The model under review builds one solid part; all positions refer to its coordinate system, in mm. A direction names the side the tool comes from. Round coordinates to 2 decimals unless told otherwise and drop trailing zeros. Order: outer loops, then holes, each group sorted by start corner. A loop starts at its lowest first (then second) coordinate and runs counter-clockwise, first axis right, second up.
1) Machinability: for faces 1 (the face through (75, 22, -3.5)), 2 (the face through (170.645, 0.454, 0.049)), which of the approach directions +Z, -Z, +X, -X, +Y, -Y give a long, thin tool a straight path to every point of the face, cutting with its end or side? Answer none if there is none.
2) To check wall thickness, follow L1, parallel to Y at x = 29.5, z = 3; L2, parallel to X at y = 0.5, z = 0. State the ranges of each line that lie inside material, in increasing order.
3) Consider section B-B (x = 38.5). Give the boundary of the cut face in (y, z).
4) Consider section C-C (z = -0.5). Give the boundary of the cut face in (x, y).
5) Consider section A-A (y = 0). Give the boundary of the cut face in (x, z), then the cut area to 3 significant figures.
6) Clearance check with a flat-ended pin moving along its axis: P1, Ø2, axis at y = -3.5, z = 2, coming from the -X side. State where the tip first meets the part, or that it passes through.
7) Mouldability with a two-part tool opening along X and no side actions: class faces 3 (the face through (76, -20.65, 0)), 4 (the face through (-22.645, -0.498, 0.049)), 5 (the face through (-20.645, -0.454, 0.049)), 6 (the face through (74, 22.65, 0)) as pulls with the +X half, pulls with the -X half, needs draft (parallel to the pull), parting line crosses it, or undercut.
from build123d import *

# Parameters (mm, degrees)
EXTRUDE_1_DEPTH = 3.5


with BuildPart() as part:
    # 草图1 → 拉伸-薄壁1 (new, symmetric)
    with BuildSketch(Plane.XY):
        with BuildLine():
            Line((150, -22.65), (0, -22.65))
            ThreePointArc((0, -22.65), (-22.65, 0), (0, 22.65))
            Line((0, 22.65), (150, 22.65))
            ThreePointArc((150, 22.65), (172.65, 0), (150, -22.65))
        make_face()
        with BuildLine():
            Line((150, -20.65), (0, -20.65))
            ThreePointArc((0, -20.65), (-20.65, 0), (0, 20.65))
            Line((0, 20.65), (150, 20.65))
            ThreePointArc((150, 20.65), (170.65, 0), (150, -20.65))
        make_face(mode=Mode.SUBTRACT)
    extrude(amount=EXTRUDE_1_DEPTH, both=True)


solid = part.part
Answer below:
1. face 1: -Z, +X, -X, +Y, -Y
1. face 2: +Z, -Z
2. L1: y = -22.65 to -20.65, 20.65 to 22.65
2. L2: x = -22.64 to -20.64, 170.64 to 172.64
3. outline: (-22.65, -3.5) - (-20.65, -3.5) - (-20.65, 3.5) - (-22.65, 3.5) - close; (20.65, -3.5) - (22.65, -3.5) - (22.65, 3.5) - (20.65, 3.5) - close
4. outline: (0, -22.65) - (150, -22.65) arc R22.65 ccw to (150, 22.65) - (0, 22.65) arc R22.65 ccw to start; hole (0, -20.65) - (150, -20.65) arc R20.65 ccw to (150, 20.65) - (0, 20.65) arc R20.65 ccw to start
5. outline: (-22.65, -3.5) - (-20.65, -3.5) - (-20.65, 3.5) - (-22.65, 3.5) - close; (170.65, -3.5) - (172.65, -3.5) - (172.65, 3.5) - (170.65, 3.5) - close
5. area: 28.0 mm2
6. P1: stops at x = -22.51
7. face 3: undercut
7. face 4: pulls with the -X half
7. face 5: undercut
7. face 6: needs draft
